from build123d import *
from OCP.BRepFilletAPI import BRepFilletAPI_MakeChamfer

# Parameters (mm, degrees)
JOURNAL_CHAMFER_0_5MM_A_SIZE  = 0.5
JOURNAL_CHAMFER_0_5MM_B_SIZE  = 0.5
BODY_EDGE_CHAMFER_3MM_SIZE    = 3
BODY_EDGE_CHAMFER_3MM_SIZE2   = 3.300188603
CENTRE_HOLE_10X59_END_A_D     = 10
CENTRE_HOLE_10X59_END_A_DEPTH = 59
CENTRE_HOLE_10X59_END_B_D     = 10
CENTRE_HOLE_10X59_END_B_DEPTH = 59


with BuildPart() as part:
    # Roller Profile Sketch → Roller Body (revolve)
    with BuildSketch(Plane.XY):
        Polygon((0, 0), (0, 12.5), (16.5, 12.5), (19.780824882, 50), (180.219175118, 50), (183.5, 12.5), (200, 12.5), (200, 0), align=None)
    revolve(axis=Axis((200, 0, 0), (-1, 0, 0)))

    # Journal Chamfer 0.5mm A
    journal_chamfer_0_5mm_a_edges = [part.edges().sort_by_distance(p)[0] for p in [
        (200, -12.5, 0),
    ]]
    chamfer(journal_chamfer_0_5mm_a_edges, length=JOURNAL_CHAMFER_0_5MM_A_SIZE)

    # Journal Chamfer 0.5mm B
    journal_chamfer_0_5mm_b_edges = [part.edges().sort_by_distance(p)[0] for p in [
        (0, -12.5, 0),
    ]]
    chamfer(journal_chamfer_0_5mm_b_edges, length=JOURNAL_CHAMFER_0_5MM_B_SIZE)

    # Body Edge Chamfer 3mm: one chamfer whose edges measure the first distance from different faces: ONE call of the kernel's chamfer builder (chamfer() names one face for all edges)
    body_edge_chamfer_3mm_edges_1 = [part.edges().sort_by_distance(p)[0] for p in [
        (180.219175118, -50, 0),
    ]]
    body_edge_chamfer_3mm_side_1 = [part.faces().sort_by_distance(p)[0] for p in [
        (100, -50, 0),
    ]]
    body_edge_chamfer_3mm_edges_2 = [part.edges().sort_by_distance(p)[0] for p in [
        (19.780824882, -50, 0),
    ]]
    body_edge_chamfer_3mm_side_2 = [part.faces().sort_by_distance(p)[0] for p in [
        (18.140412441, -31.25, 0),
    ]]
    body_edge_chamfer_3mm = BRepFilletAPI_MakeChamfer(part.part.solid().wrapped)
    for e in body_edge_chamfer_3mm_edges_1:
        body_edge_chamfer_3mm.Add(BODY_EDGE_CHAMFER_3MM_SIZE, BODY_EDGE_CHAMFER_3MM_SIZE2, e.wrapped, body_edge_chamfer_3mm_side_1[0].wrapped)  # the first distance lies on this face
    for e in body_edge_chamfer_3mm_edges_2:
        body_edge_chamfer_3mm.Add(BODY_EDGE_CHAMFER_3MM_SIZE, BODY_EDGE_CHAMFER_3MM_SIZE2, e.wrapped, body_edge_chamfer_3mm_side_2[0].wrapped)  # the first distance lies on this face
    add(Compound.cast(body_edge_chamfer_3mm.Shape()), mode=Mode.REPLACE)

    # Centre Hole Ø10x59 End A
    with Locations(Plane(origin=(200, 0, 0), x_dir=(0, 0, -1), z_dir=(1, 0, 0))):
        with Locations((0, 0)):
            Hole(CENTRE_HOLE_10X59_END_A_D / 2, depth=CENTRE_HOLE_10X59_END_A_DEPTH)

    # Centre Hole Ø10x59 End B
    with Locations(Plane.ZY):
        with Locations((0, 0)):
            Hole(CENTRE_HOLE_10X59_END_B_D / 2, depth=CENTRE_HOLE_10X59_END_B_DEPTH)


solid = part.part
Part model, mm, in its own coordinate system. A direction names the side the tool comes from. Coordinates: 2 decimals unless noted, no trailing zeros. Order: outer loops, then holes, each group sorted by start corner. A loop starts at its lowest first (then second) coordinate and runs counter-clockwise, first axis right, second up.
(1) Tool access for faces 5 (the face through (29.91, -4.88, 1.08)), 6 (the face through (101.23, 23.07, 44.36)), 7 (the face through (191.612, 11.923, -3.755)): list every direction of +Z, -Z, +X, -X, +Y, -Y with a clear straight run to the whole face (end or side of a thin tool).
Check sheet entries:
face 5: -X
face 6: +X, -X
face 7: +X
(2) Slice it at B-B, the plane x = 102.5. Write the cut outline in (y, z).
Check sheet entries:
outline: circle Ø100 at (0, 0)
(3) Probe L1, parallel to Y at x = 38.5, z = 0; L2, parallel to Z at x = 61, y = 0; L3, parallel to Y at x = 159, z = -2.5. List the from-to ranges inside material, lowest first.
Check sheet entries:
L1: y = -50 to -5, 5 to 50
L2: z = -50 to 50
L3: y = -49.94 to -4.33, 4.33 to 49.94
(4) Pull direction Y, two halves, no side cores. Call faces 1 (the face through (59, 0, 0)), 2 (the face through (200, 5.2, -0.2)), 3 (the face through (8.612, 11.923, -3.755)), 4 (the face through (141, 0, 0)): pulls with the +Y half, pulls with the -Y half, needs draft (parallel to the pull), parting line crosses it, or undercut.
Check sheet entries:
face 1: undercut
face 2: needs draft
face 3: parting line crosses it
face 4: undercut
(5) Pin check, flat tips, straight feed: pin 1 Ø10 at (x, z) = (146.5, -5) entering from -Y; pin 2 Ø5 at (x, y) = (80, -33.5) entering from -Z; pin 3 Ø5 at (x, z) = (91, 16) entering from +Y; pin 4 Ø12 at (x, z) = (116.5, 16) entering from +Y. Stop position of each tip, or through.
Check sheet entries:
pin 1: stops at y = -50
pin 2: stops at z = -39.23
pin 3: stops at y = 48.14
pin 4: stops at y = 48.99
(6) Slice it at A-A, the plane x = 50.5. Write the cut outline in (y, z), and give its area (3 significant figures).
Check sheet entries:
outline: circle Ø100 at (0, 0); hole circle Ø10 at (0, 0)
area: 7,780 mm2
